Source: CAD feature listing. Evaluate the final solid. Frame: model axes, mm. A direction names the side the tool comes from. Give positions to 0.01 mm unless a question says otherwise; leave off trailing zeros. Write each loop counter-clockwise with the first axis right and the second up, starting at its lowest first coordinate (ties: lowest second). Pieces come first, ordered by that corner, then holes. Notation, with made-up numbers: M 27,54 L 82,54 A19 ccw 82,82 Z; hole C 82,11 d8. An arc over 180 degrees is marked long. Return JSON: item names as keys, results as strings.
```python
from build123d import *

# Parameters (mm, degrees)
BASE_BLOCK_DEPTH          = 25
UPRIGHT_BLOCK_DEPTH       = 18
SIDE_TAB_SKETCH_W         = 12
SIDE_TAB_SKETCH_H         = 32
SIDE_TAB_DEPTH            = 42
FRONT_PLATE_SKETCH_W      = 52
FRONT_PLATE_SKETCH_H      = 42
FRONT_PLATE_DEPTH         = 10
FRONT_PLATE_HOLE_SKETCH_R = 9
FRONT_PLATE_HOLE_DEPTH    = 10
SIDE_TAB_HOLES_SKETCH_R   = 4
SIDE_TAB_HOLES_2X_DEPTH   = 12
TRIANGULAR_GUSSET_DEPTH   = 18


with BuildPart() as part:
    # Base Block Sketch → Base Block (new body)
    with BuildSketch(Plane.XY):
        Polygon((0, 0), (112, 0), (112, 32), (89, 78), (0, 78), align=None)
    extrude(amount=BASE_BLOCK_DEPTH)

    # Upright Block Sketch → Upright Block (add)
    with BuildSketch(Plane.ZY):
        Polygon((71, 36), (25, 36), (25, 78), (83, 78), (83, 36), align=None)
    extrude(amount=-UPRIGHT_BLOCK_DEPTH)

    # Side Tab Sketch → Side Tab (add)
    with BuildSketch(Plane.ZY):
        with Locations((26, 62)):
            Rectangle(SIDE_TAB_SKETCH_W, SIDE_TAB_SKETCH_H)
    extrude(amount=SIDE_TAB_DEPTH)

    # Front Plate Sketch → Front Plate (add)
    with BuildSketch(Plane.XY.offset(83)):
        with Locations((44, 57)):
            Rectangle(FRONT_PLATE_SKETCH_W, FRONT_PLATE_SKETCH_H)
    extrude(amount=-FRONT_PLATE_DEPTH)

    # Front Plate Hole Sketch → Front Plate Hole (cut)
    with BuildSketch(Plane.XY.offset(83)):
        with Locations((50, 57)):
            Circle(FRONT_PLATE_HOLE_SKETCH_R)
    extrude(amount=-FRONT_PLATE_HOLE_DEPTH, mode=Mode.SUBTRACT)

    # Side Tab Holes Sketch → Side Tab Holes 2x (cut)
    with BuildSketch(Plane.XY.offset(32)):
        with Locations((-31, 68)):
            Circle(SIDE_TAB_HOLES_SKETCH_R)
        with Locations((-19, 58)):
            Circle(SIDE_TAB_HOLES_SKETCH_R)
    extrude(amount=-SIDE_TAB_HOLES_2X_DEPTH, mode=Mode.SUBTRACT)

    # Gusset Sketch → Triangular Gusset (add)
    with BuildSketch(Plane.ZY):
        Polygon((25, 36), (73, 36), (25, 8), align=None)
    extrude(amount=-TRIANGULAR_GUSSET_DEPTH)


solid = part.part
```
1) Line query: line 1 (Y direction, x = -31, z = 26.5); line 2 (Z direction, x = 59.5, y = 45.5); line 3 (Y direction, x = 50, z = 77.5). Output: solid intervals per line, ascending. Write a range as [from, to].
Numbers:
{"line 1": "y = [46, 64], [72, 78]", "line 2": "z = [0, 25], [73, 83]", "line 3": "y = [36, 48], [66, 78]"}
2) Cut plane D-D, the plane x = -31. Return the cut outline in (y, z), then the cut area to 3 significant figures.
Numbers:
{"outline": "M 46,20 L 64,20 L 64,32 L 46,32 Z; M 72,20 L 78,20 L 78,32 L 72,32 Z", "area": "288 mm²"}
3) Contact query for flat-ended pins moving along their axis: pin 1 Ø5 at (x, y) = (78.5, 41) entering from +Z; pin 2 Ø6.5 at (x, y) = (-31, 68) entering from +Z; pin 3 Ø13 at (x, z) = (-19.5, 28) entering from -Y; pin 4 Ø3 at (y, z) = (66, 75.5) entering from +X. Output: stop coordinate, or through.
Numbers:
{"pin 1": "stops at z = 25", "pin 2": "passes through", "pin 3": "stops at y = 46", "pin 4": "stops at x = 70"}
4) Cut plane C-C, the plane z = 11. Return the cut outline in (x, y).
Numbers:
{"outline": "M 0,0 L 112,0 L 112,32 L 89,78 L 0,78 Z"}
5) Set-up query: faces 1 (the face through (-21, 62, 20)), 2 (the face through (38, 57, 73)), 3 (the face through (42.86, 51.52, 78.07)), 4 (the face through (-21, 46, 26)), 5 (the face through (70, 57, 78)). Return all of +Z, -Z, +X, -X, +Y, -Y with unobstructed straight access to the full face (end or side cutting, diameter ignored); none if empty.
Numbers:
{"face 1": "-Z, -X, +Y, -Y", "face 2": "+X, +Y, -Y", "face 3": "+Z", "face 4": "+Z, -Z, -X, -Y", "face 5": "+Z, +X, +Y, -Y"}
6) Draft query along Y for faces 6 (the face through (35, 36, 78)), 7 (the face through (-31.867, 64.095, 26.084)), 8 (the face through (-21, 62, 32)). Return one class per face: released by +Y, released by -Y, zero draft, split by the parting line, or undercut.
Numbers:
{"face 6": "released by -Y", "face 7": "undercut", "face 8": "zero draft"}
7) Cut plane B-B, the plane x = 65. Return the cut outline in (y, z).
Numbers:
{"outline": "M 0,0 L 78,0 L 78,25 L 0,25 Z; M 36,73 L 78,73 L 78,83 L 36,83 Z"}
8) Cut plane A-A, the plane y = 68. Return the cut outline in (x, z), then the cut area to 3 significant figures.
Numbers:
{"outline": "M -42,20 L -35,20 L -35,32 L -42,32 Z; M -27,20 L 0,20 L 0,0 L 94,0 L 94,25 L 18,25 L 18,73 L 70,73 L 70,83 L 0,83 L 0,32 L -27,32 Z", "area": "4,320 mm²"}
